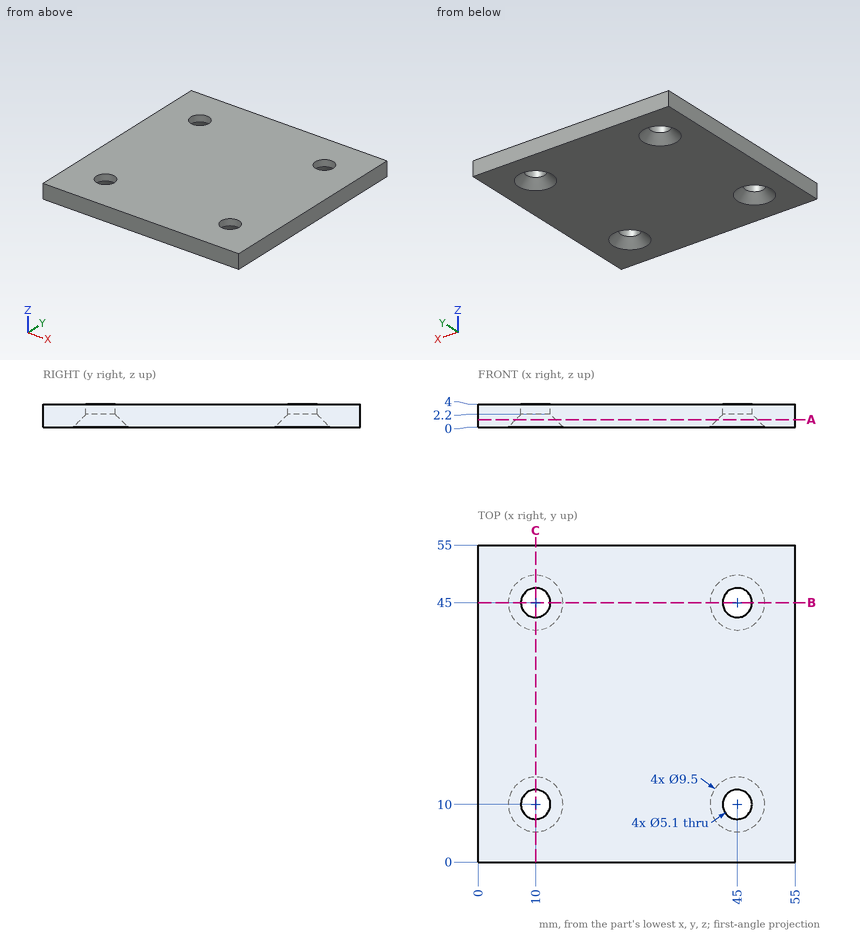
Drawing for the job (mm, zero at the part's lowest x, y, z). Give positions to 0.01 mm unless a question says otherwise; leave off trailing zeros. Loops run counter-clockwise (first coordinate to the right, second up) from the corner with the lowest first, then second, coordinate; pieces in that order, holes last. Notation, with made-up numbers: M -22.5,-31 L 18.5,-31 A23 ccw 18.5,-10 Z; hole C 82,-20.75 d7. An arc over 180 degrees is marked long. One line per question, with ' | ' between items. Start each with the question number.
1. Probe L1, parallel to Y at x = 45, z = 3.4; L2, parallel to X at y = 49, z = 0.25; L3, parallel to X at y = 48, z = 1.2. List the from-to ranges inside material, lowest first. Write a range as from..to.
2. Saw through at A-A on z = 1.3. Give the cut face in (x, y).
3. Saw through at B-B on y = 45. Give the cut face in (x, z), plus the area to 3 significant figures.
Result sheet:
1) L1: y = 0..7.45, 12.55..42.45, 47.55..55 | L2: x = 0..7.94, 12.06..42.94, 47.06..55 | L3: x = 0..8.1, 11.9..43.1, 46.9..55
2) outline: M 0,0 L 55,0 L 55,55 L 0,55 Z; hole C 10,10 d6.9; hole C 10,45 d6.9; hole C 45,10 d6.9; hole C 45,45 d6.9
3) outline: M 0,0 L 5.25,0 L 7.45,2.2 L 7.45,4 L 0,4 Z; M 12.55,2.2 L 14.75,0 L 40.25,0 L 42.45,2.2 L 42.45,4 L 12.55,4 Z; M 47.55,2.2 L 49.75,0 L 55,0 L 55,4 L 47.55,4 Z | area: 170 mm^2
